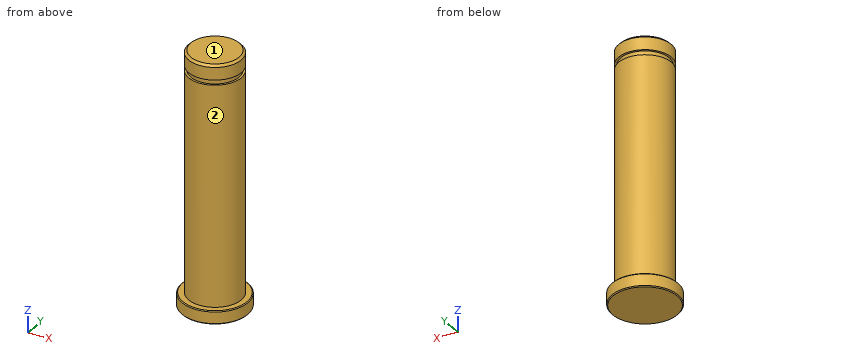
from build123d import *

# Parameters (mm, degrees)
SKETCH1_R           = 7.5
BOSS_EXTRUDE1_DEPTH = 3
SKETCH2_R           = 6
BOSS_EXTRUDE2_DEPTH = 54.5
CHAMFER1_SIZE       = 0.2
SKETCH3_W           = 0.5
SKETCH3_H           = 1.15
CHAMFER2_SIZE       = 0.5


with BuildPart() as part:
    # Sketch1 → Boss-Extrude1 (new body)
    with BuildSketch(Plane.XY):
        Circle(SKETCH1_R)
    extrude(amount=BOSS_EXTRUDE1_DEPTH)

    # Sketch2 → Boss-Extrude2 (add)
    with BuildSketch(Plane.XY.offset(3)):
        Circle(SKETCH2_R)
    extrude(amount=BOSS_EXTRUDE2_DEPTH)

    # Chamfer1
    chamfer1_edges = [part.edges().sort_by_distance(p)[0] for p in [
        (-7.5, 0, 0),
        (-7.5, 0, 3),
    ]]
    chamfer(chamfer1_edges, length=CHAMFER1_SIZE)

    # Sketch3 → Cut-Revolve1 (revolve, cut)
    with BuildSketch(Plane(origin=(0, 0, 0), x_dir=(1, 0, 0), z_dir=(0, 1, 0)), mode=Mode.PRIVATE) as cut_revolve1_sk:
        with Locations((-5.75, -53.575)):
            Rectangle(SKETCH3_W, SKETCH3_H)
    revolve(cut_revolve1_sk.sketch.rotate(Axis((0, 0, 57.5), (0, 0, -1)), 180), axis=Axis((0, 0, 57.5), (0, 0, -1)), mode=Mode.SUBTRACT)

    # Chamfer2
    chamfer2_edges = [part.edges().sort_by_distance(p)[0] for p in [
        (-6, 0, 57.5),
    ]]
    chamfer(chamfer2_edges, length=CHAMFER2_SIZE)


solid = part.part
Verification items for the finished model (mm, model axes). Face numbers are marked on the shaded views. A direction names the side the tool comes from. Give positions to 0.01 mm unless a question says otherwise; leave off trailing zeros. Order: outer loops, then holes, each group sorted by start corner. A loop starts at its lowest first (then second) coordinate and runs counter-clockwise, first axis right, second up. Notation, with made-up numbers: M 17.5,10.5 L 31.5,10.5 A18 ccw 31.5,27.5 Z; hole C -11,22 d9. An arc over 180 degrees is marked long. Use one line per item in the form item = value. Start each with the question number.
Q1. Access from +Z, -Z, +X, -X, +Y, -Y to the whole of each face (thin tool, end or side, straight path). Record for the marked faces 1 and 2.
Q2. Go/stop test with flat-tipped pins: pin 1 Ø5 at (x, z) = (1, 48.5) entering from -Y; pin 2 Ø1 at (x, z) = (-3, 7.5) entering from -Y; pin 3 Ø6 at (y, z) = (2.5, 10) entering from +X. Record where each tip stops, or that it passes through.
Q3. Section check A-A (x = 0). Enter the section's corners in (y, z), then the cut area to 3 significant figures.
Q4. Section check C-C (z = 5.5). Enter the section's corners in (x, y).
Q5. Scan lines: line 1 along Z through (x, y) = (-2.5, 5.5); line 2 along Y through (x, z) = (0, 48); line 3 along Y through (x, z) = (3.75, 21). Record each from-to range of solid material in increasing order. Write a range as [from, to].
Evaluation:
q1.face_1 = +Z, +X, -X, +Y, -Y
q1.face_2 = +Z
q2.pin_1 = -6
q2.pin_2 = -5.45
q2.pin_3 = 6
q3.outline = M -7.5,0.2 L -7.3,0 L 7.3,0 L 7.5,0.2 L 7.5,2.8 L 7.3,3 L 6,3 L 6,53 L 5.5,53 L 5.5,54.15 L 6,54.15 L 6,57 L 5.5,57.5 L -5.5,57.5 L -6,57 L -6,54.15 L -5.5,54.15 L -5.5,53 L -6,53 L -6,3 L -7.3,3 L -7.5,2.8 Z
q3.area = 698 mm2
q4.outline = C 0,0 d12
q5.line_1 = [0, 3]
q5.line_2 = [-6, 6]
q5.line_3 = [-4.68, 4.68]
